```python
from build123d import *

# Parameters (mm, degrees)
BASE_PROFILE_SKETCH_W  = 40
BASE_PROFILE_SKETCH_H  = 46
BASE_BLOCK_DEPTH       = 38
BOTTOM_STEP_SKETCH_W   = 8
BOTTOM_STEP_SKETCH_H   = 8
BOTTOM_STEP_CUT_DEPTH  = 49.713447835
CORNER_NOTCH_SKETCH_W  = 8
CORNER_NOTCH_SKETCH_H  = 8
CORNER_NOTCH_8X8_DEPTH = 49.713447835
V_GROOVE_CUT_DEPTH     = 46
SLOT_CUT_8X8_DEPTH     = 46
SIDE_TRIM_SKETCH_W     = 22.317279544
SIDE_TRIM_SKETCH_H     = 4.669832792
SIDE_TRIM_CUT_DEPTH    = 46


with BuildPart() as part:
    # Base Profile Sketch → Base Block (new body)
    with BuildSketch(Plane.XY):
        Rectangle(BASE_PROFILE_SKETCH_W, BASE_PROFILE_SKETCH_H)
    extrude(amount=BASE_BLOCK_DEPTH)

    # Bottom Step Sketch → Bottom Step Cut (cut, through all)
    with BuildSketch(Plane.XY.offset(38)):
        with Locations((-16, -19)):
            Rectangle(BOTTOM_STEP_SKETCH_W, BOTTOM_STEP_SKETCH_H)
    extrude(amount=-BOTTOM_STEP_CUT_DEPTH, mode=Mode.SUBTRACT)

    # Corner Notch Sketch → Corner Notch 8x8 (cut, through all)
    with BuildSketch(Plane.XY.offset(38)):
        with Locations((16, -19)):
            Rectangle(CORNER_NOTCH_SKETCH_W, CORNER_NOTCH_SKETCH_H)
    extrude(amount=-CORNER_NOTCH_8X8_DEPTH, mode=Mode.SUBTRACT)

    # V-Groove Profile Sketch → V-Groove Cut (cut, symmetric)
    with BuildSketch(Plane(origin=(0, 0, 0), x_dir=(0, 0, -1), z_dir=(1, 0, 0))):
        Polygon((-38, 0), (-30.842105263, 0), (-26, 23), (-38, 23), align=None)
        Polygon((-12, 23), (-7.157894737, 0), (0, 0), (0, 23), align=None)
    extrude(amount=V_GROOVE_CUT_DEPTH, both=True, mode=Mode.SUBTRACT)

    # Slot Sketch → Slot Cut 8x8 (cut, symmetric)
    with BuildSketch(Plane(origin=(0, -1.442970822, 6.854111406), x_dir=(-1, 0, 0), z_dir=(0, 0.206010481049842, -0.9785497849867492))):
        Polygon((-7.180041029, 14.15108932), (0.819958971, 14.15108932), (8.819958971, 14.15108932), (11.331109989, 24.978770827), (-10.986169555, 24.978770827), align=None)
    extrude(amount=SLOT_CUT_8X8_DEPTH, both=True, mode=Mode.SUBTRACT)

    # Side Trim Sketch → Side Trim Cut (cut, symmetric)
    with BuildSketch(Plane(origin=(0, -1.442970822, 6.854111406), x_dir=(-1, 0, 0), z_dir=(0, 0.206010481049842, -0.9785497849867492))):
        with Locations((0.172470217, 27.313687223)):
            Rectangle(SIDE_TRIM_SKETCH_W, SIDE_TRIM_SKETCH_H)
    extrude(amount=SIDE_TRIM_CUT_DEPTH, both=True, mode=Mode.SUBTRACT)


solid = part.part
```
Read the model definition and answer for the solid it produces. Units are mm, in the model's axes. A direction names the side the tool comes from. Coordinates: 2 decimals unless noted, no trailing zeros. Write each loop counter-clockwise with the first axis right and the second up, starting at its lowest first coordinate (ties: lowest second). Pieces come first, ordered by that corner, then holes. Notation, with made-up numbers: (79, 76.5) - (115, 76.5) arc R28 ccw to (115, 107.5) - close; hole circle Ø3 at (-16.75, 82). An arc over 180 degrees is marked (long way). Answer as a JSON object with one key per item and string values. Group by question number.
1. A cutting plane is placed at C-C (z = 3). Determine the outline of the cut face in (x, y).
2. Which of the six approach directions +Z, -Z, +X, -X, +Y, -Y give full straight-line access (tool end or side, diameter ignored) to faces 4 (the flat face through (-16, -15, 19)), 5 (the flat face through (-10.058, 15.623, 20.393)), 6 (the flat face through (0, 0, 34)), 7 (the flat face through (12, -19, 19))?
3. Each of these flat-tipped pins is pushed along its axis until it touches: P1, Ø4, axis at x = 16, z = 24.5, coming from the -Y side; P2, Ø3, axis at x = 8, y = 7, coming from the -Z side; P3, Ø5, axis at x = 15, y = 6.5, coming from the +Z side; P4, Ø6, axis at y = 17.5, z = 33, coming from the -X side. Where does it stop, or does it pass through?
4. A cutting plane is placed at B-B (x = -0.5). Determine the outline of the cut face in (y, z).
5. A cutting plane is placed at D-D (z = 22.5). Determine the outline of the cut face in (x, y).
6. The mould has two halves that part along X. Classify faces 1 (the flat face through (-12, -19, 19)), 2 (the flat face through (-16, 23, 19)), 3 (the flat face through (-11.331, 22, 21)): +X half, -X half, draft (parallel to the pull), parting line (faces both ways), or undercut.
7. A cutting plane is placed at A-A (y = 17). Determine the outline of the cut face in (x, z), plus the area to 3 significant figures.
8. Consider L1, parallel to Y at x = 14.5, z = 24.5; L2, parallel to X at y = -17, z = 26.5; L3, parallel to X at y = 11, z = 24.5 (3 decimals). Determine where each line is inside the solid, lowest interval first. Write a range as [from, to].
Worked out:
{
 "1": {"outline": "(-20, -15) - (-12, -15) - (-12, -23) - (12, -23) - (12, -15) - (20, -15) - (20, 0) - (-20, 0) - close"},
 "2": {"face 4": "+Z, -Z, -X, -Y", "face 5": "+Z, +Y", "face 6": "+Z, +X, -X, +Y", "face 7": "+Z, -Z, +X, -Y"},
 "3": {"P1": "stops at y = -15", "P2": "stops at z = 8.32", "P3": "stops at z = 30", "P4": "passes through"},
 "4": {"outline": "(-23, 0) - (0, 0) - (0, 7.16) - (12.4, 9.77) - (8.34, 29.09) - (0, 30.84) - (0, 38) - (-23, 38) - close"},
 "5": {"outline": "(-20, -15) - (-12, -15) - (-12, -23) - (12, -23) - (12, -15) - (20, -15) - (20, 23) - (10.99, 23) - (10.99, 20.79) - (7.18, 9.72) - (-8.82, 9.72) - (-11.33, 20.79) - (-11.33, 23) - (-20, 23) - close"},
 "6": {"face 1": "-X half", "face 2": "draft", "face 3": "undercut"},
 "7": {"outline": "(-20, 10.74) - (-9.91, 10.74) - (-10.7, 27.26) - (-20, 27.26) - close; (8.83, 10.74) - (20, 10.74) - (20, 27.26) - (10.03, 27.26) - close", "area": "335 mm²"},
 "8": {"L1": "y = [-15, 23]", "L2": "x = [-12, 12]", "L3": "x = [-20, -9.205], [7.764, 20]"}
}
